CAD build for the part. Positions are in the model's coordinates, mm. Face numbers are marked on the shaded views. A direction names the side the tool comes from. Coordinates: 2 decimals unless noted, no trailing zeros. Loops run counter-clockwise (first coordinate to the right, second up) from the corner with the lowest first, then second, coordinate; pieces in that order, holes last. Notation, with made-up numbers: (83.5, 12.25) - (116.5, 12.25) arc R25 ccw to (116.5, 35.25) - close; hole circle Ø6 at (21, 24.5). An arc over 180 degrees is marked (long way). Put each result on its own line as item: value.
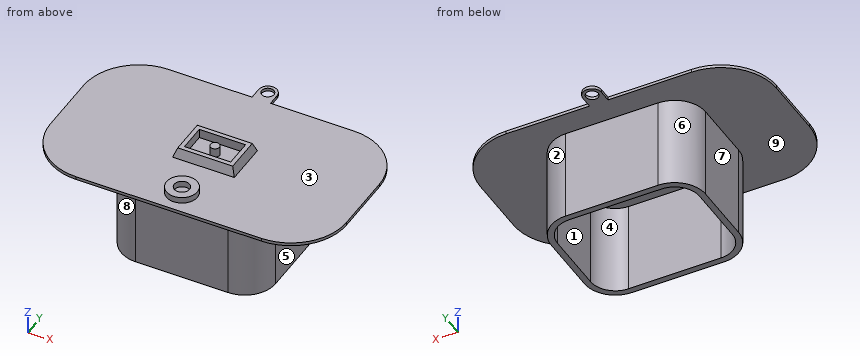
```python
from build123d import *

# Parameters (mm, degrees)
SKETCH1_R           = 2
BOSS_EXTRUDE1_DEPTH = 1
SKETCH2_W           = 20
SKETCH2_H           = 14
BOSS_EXTRUDE2_DEPTH = 3
BOSS_EXTRUDE2_TAPER = 20
SKETCH3_W           = 15
SKETCH3_H           = 9
SKETCH3_R           = 1.5
CUT_EXTRUDE1_DEPTH  = 3
SKETCH4_W           = 50
SKETCH4_H           = 40
SKETCH4_W_2         = 46
SKETCH4_H_2         = 36
BOSS_EXTRUDE3_DEPTH = 30
SKETCH5_R           = 5
SKETCH5_R_2         = 2.5
BOSS_EXTRUDE4_DEPTH = 2
FILLET1_R           = 8
FILLET2_R           = 10


with BuildPart() as part:
    # Sketch1 → Boss-Extrude1 (new body)
    with BuildSketch(Plane.XY):
        with BuildLine():
            Line((-3, 28), (-3, 32))
            ThreePointArc((-3, 32), (0, 35), (3, 32))
            Line((3, 32), (3, 28))
            Line((3, 28), (30, 28))
            ThreePointArc((30, 28), (42.727922061, 22.727922061), (48, 10))
            Line((48, 10), (48, -10))
            ThreePointArc((48, -10), (42.727922061, -22.727922061), (30, -28))
            Line((30, -28), (-30, -28))
            ThreePointArc((-30, -28), (-42.727922061, -22.727922061), (-48, -10))
            Line((-48, -10), (-48, 10))
            ThreePointArc((-48, 10), (-42.727922061, 22.727922061), (-30, 28))
            Line((-30, 28), (-3, 28))
        make_face()
        with Locations((0, 32)):
            Circle(SKETCH1_R, mode=Mode.SUBTRACT)
    extrude(amount=BOSS_EXTRUDE1_DEPTH)

    # Sketch2 → Boss-Extrude2 (add)
    with BuildSketch(Plane.XY.offset(1)):
        Rectangle(SKETCH2_W, SKETCH2_H)
    extrude(amount=BOSS_EXTRUDE2_DEPTH, taper=BOSS_EXTRUDE2_TAPER)

    # Sketch3 → Cut-Extrude1 (cut)
    with BuildSketch(Plane.XY.offset(4)):
        Rectangle(SKETCH3_W, SKETCH3_H)
        Circle(SKETCH3_R, mode=Mode.SUBTRACT)
    extrude(amount=-CUT_EXTRUDE1_DEPTH, mode=Mode.SUBTRACT)

    # Sketch4 → Boss-Extrude3 (add)
    with BuildSketch(Plane(origin=(0, 0, 0), x_dir=(-1, 0, 0), z_dir=(0, 0, -1))):
        Rectangle(SKETCH4_W, SKETCH4_H)
        Rectangle(SKETCH4_W_2, SKETCH4_H_2, mode=Mode.SUBTRACT)
    extrude(amount=BOSS_EXTRUDE3_DEPTH)

    # Sketch5 → Boss-Extrude4 (add)
    with BuildSketch(Plane.XY.offset(1)):
        with Locations((0, -20)):
            Circle(SKETCH5_R)
        with Locations((0, -20)):
            Circle(SKETCH5_R_2, mode=Mode.SUBTRACT)
    extrude(amount=BOSS_EXTRUDE4_DEPTH)

    # Fillet1
    fillet1_edges = [part.edges().sort_by_distance(p)[0] for p in [
        (-23, 18, -15),
        (23, 18, -15),
        (23, -18, -15),
        (-23, -18, -15),
    ]]
    fillet(fillet1_edges, radius=FILLET1_R)

    # Fillet2
    fillet2_edges = [part.edges().sort_by_distance(p)[0] for p in [
        (-25, -20, -15),
        (-25, 20, -15),
        (25, 20, -15),
        (25, -20, -15),
    ]]
    fillet(fillet2_edges, radius=FILLET2_R)


solid = part.part
```
Q1. Mould opens along X. For the marked faces 1, 2, 3 and 4 say: +X half, -X half, draft (parallel to the pull), parting line (faces both ways), or undercut.
Determined:
face 1: undercut
face 2: +X half
face 3: draft
face 4: undercut
Q2. Slice it at C-C, the plane x = -32. Give the cut face in (y, z), then the cut area to 3 significant figures.
Determined:
outline: (-27.89, 0) - (27.89, 0) - (27.89, 1) - (-27.89, 1) - close
area: 55.8 mm2
Q3. Pin check, flat tips, straight feed: pin 1 Ø12 at (x, y) = (32.5, 2.5) entering from +Z; pin 2 Ø4 at (y, z) = (-19, -19) entering from -X; pin 3 Ø8 at (y, z) = (28, -1) entering from +X; pin 4 Ø3 at (x, y) = (0, 32) entering from -Z. Stop position of each tip, or through.
Determined:
pin 1: z = 1
pin 2: x = -22.14
pin 3: x = 41.15
pin 4: through
Q4. Slice it at B-B, the plane y = 0. Give the cut face in (x, z), then the cut area to 3 significant figures.
Determined:
outline: (-48, 0) - (-25, 0) - (-25, -30) - (-23, -30) - (-23, 0) - (23, 0) - (23, -30) - (25, -30) - (25, 0) - (48, 0) - (48, 1) - (10, 1) - (8.91, 4) - (7.5, 4) - (7.5, 1) - (1.5, 1) - (1.5, 4) - (-1.5, 4) - (-1.5, 1) - (-7.5, 1) - (-7.5, 4) - (-8.91, 4) - (-10, 1) - (-48, 1) - close
area: 237 mm2
Q5. Slice it at A-A, the plane z = -8. Give the cut face in (x, y), then the cut area to 3 significant figures.
Determined:
outline: (-25, -10) arc R10 ccw to (-15, -20) - (15, -20) arc R10 ccw to (25, -10) - (25, 10) arc R10 ccw to (15, 20) - (-15, 20) arc R10 ccw to (-25, 10) - close; hole (-23, -10) arc R8 ccw to (-15, -18) - (15, -18) arc R8 ccw to (23, -10) - (23, 10) arc R8 ccw to (15, 18) - (-15, 18) arc R8 ccw to (-23, 10) - close
area: 313 mm2
Q6. Tool access for the marked faces 5, 6, 7, 8 and 9: list every direction of +Z, -Z, +X, -X, +Y, -Y with a clear straight run to the whole face (end or side of a thin tool).
Determined:
face 5: -Z, +X, +Y, -Y
face 6: -Z, -X, +Y
face 7: -Z, -X, +Y, -Y
face 8: -Z, -X, -Y
face 9: -Z
Q7. Wall check: L1, parallel to Y at x = 0, z = 2; L2, parallel to Y at x = -13.5, z = -24; L3, parallel to X at y = 7.5, z = -18.5. Give the ranges that are in metal, low to high. Write a range as from..to.
Determined:
L1: -25..-22.5, -17.5..-15, -6.64..-4.5, -1.5..1.5, 4.5..6.64
L2: -20..-18, 18..20
L3: -25..-23, 23..25
